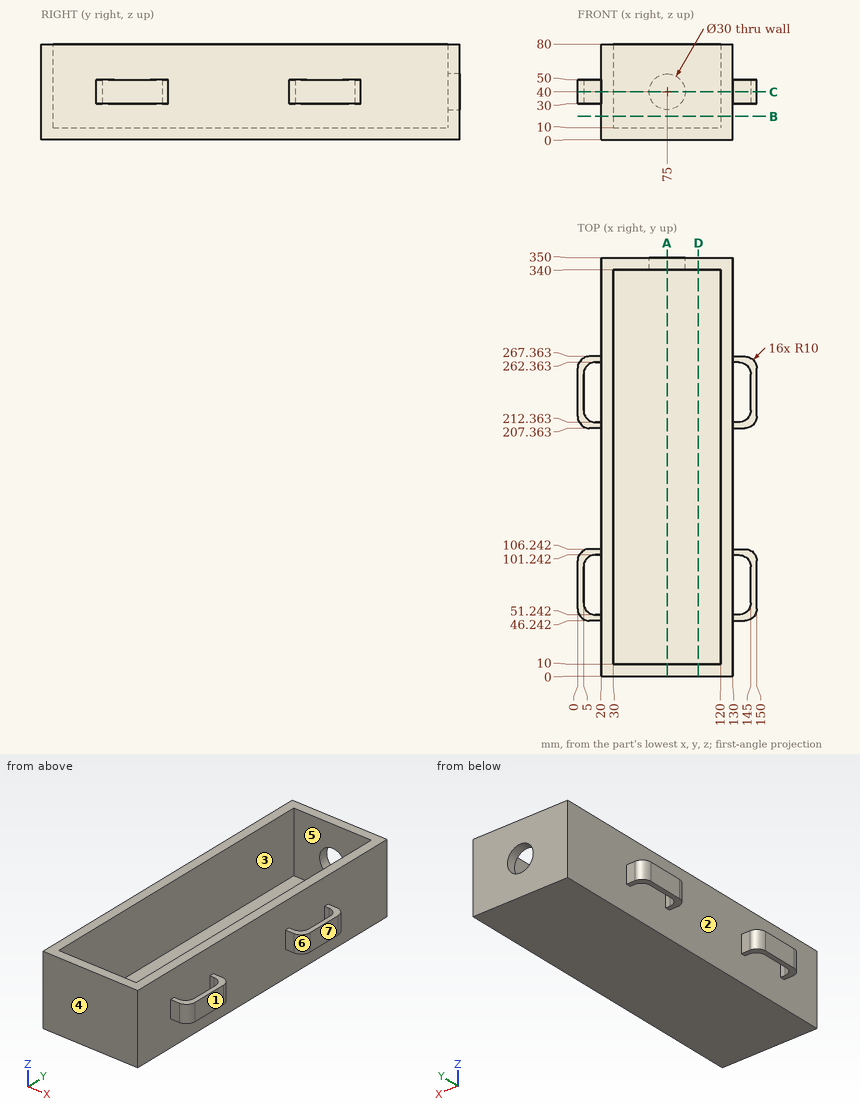
Could you check a few things on this drawing? It's one solid part, dimensions in mm from its lowest x, y, z. A direction names the side the tool comes from. Coordinates: 2 decimals unless noted, no trailing zeros. Order: outer loops, then holes, each group sorted by start corner. A loop starts at its lowest first (then second) coordinate and runs counter-clockwise, first axis right, second up.
1) Imagine slicing it at C-C on z = 40. State how many separate pieces and enclosed holes the cut face has, and give its area (3 significant figures).
2) Which directions (+Z, -Z, +X, -X, +Y, -Y) give clear straight access to the entire face, cutting with the end or side of a thin tool? Please do the marked faces 5, 6 and 7.
3) Imagine slicing it at B-B on z = 19.5. List the corners of the cut face in (x, y) for me.
4) Will these pins go through, and if not, where does the flat tip stop? pin 1 (3 mm diameter, centred on x = 134.5, z = 39.5, fed in from +Y); pin 2 (1 mm diameter, centred on y = 55.5, z = 69.5, fed in from +X); pin 3 (16 mm diameter, centred on x = 8.5, y = 224.5, fed in from -Z).
5) We'd pull the mould along Y, two halves only. Please class the marked faces 1, 2, 3 and 4: +Y half, -Y half, draft (parallel to the pull), parting line (faces both ways), or undercut.
6) Imagine slicing it at D-D on x = 101. List the corners of the cut face in (y, z) for me.
7) I need wall thicknesses on line 1 (Y direction, x = 95, z = 49); line 2 (X direction, y = 347.25, z = 40); line 3 (X direction, y = 275, z = 55). Which ranges of each line are inside material? Lowest first, please.
8) Imagine slicing it at A-A on x = 75. List the corners of the cut face in (y, z) for me.
Response values:
1. separate pieces: 1
1. enclosed holes: 4
1. area: 10,300 mm2
2. face 5: +Z
2. face 6: +Z, -Z, +X
2. face 7: +Z, -Z, +X, +Y, -Y
3. outline: (20, 0) - (130, 0) - (130, 350) - (20, 350) - close; hole (30, 10) - (120, 10) - (120, 340) - (30, 340) - close
4. pin 1: stops at y = 267.36
4. pin 2: stops at x = 130
4. pin 3: stops at z = 30
5. face 1: draft
5. face 2: undercut
5. face 3: undercut
5. face 4: -Y half
6. outline: (0, 0) - (350, 0) - (350, 80) - (340, 80) - (340, 10) - (10, 10) - (10, 80) - (0, 80) - close
7. line 1: y = 0 to 10, 340 to 350
7. line 2: x = 20 to 60, 90 to 130
7. line 3: x = 20 to 30, 120 to 130
8. outline: (0, 0) - (350, 0) - (350, 25) - (340, 25) - (340, 10) - (10, 10) - (10, 80) - (0, 80) - close; (340, 55) - (350, 55) - (350, 80) - (340, 80) - close
